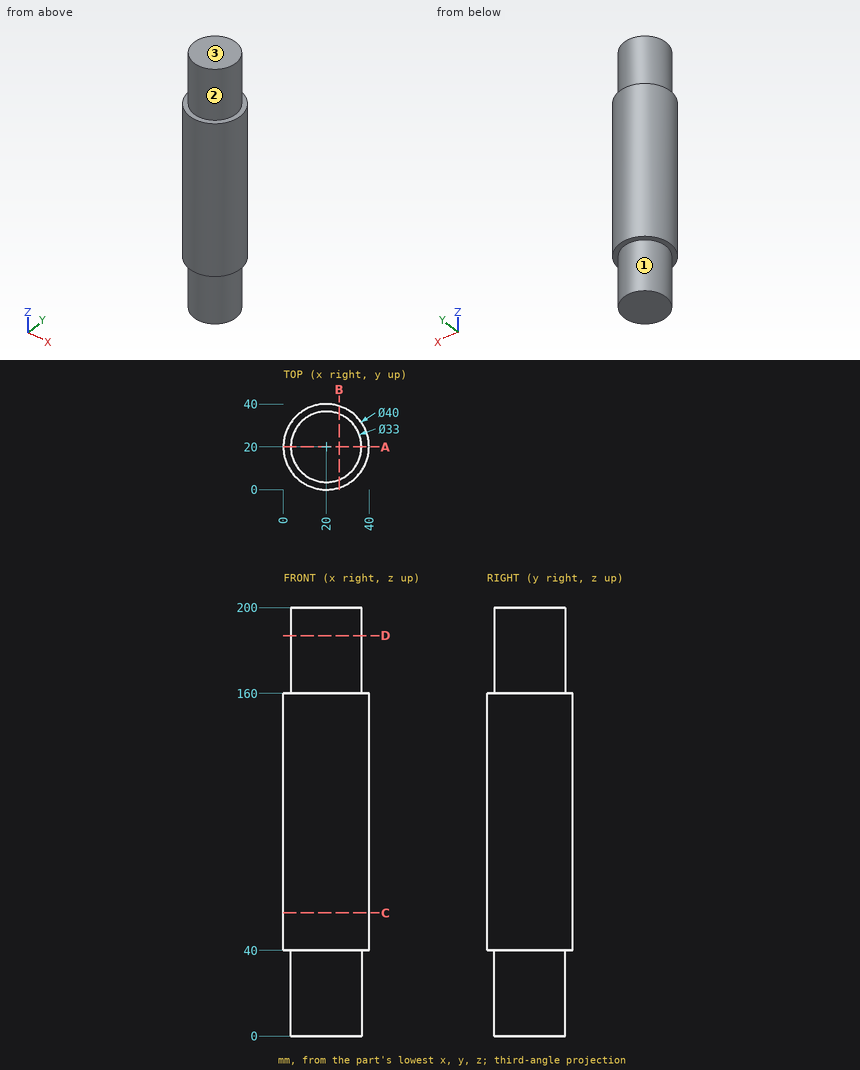
Input: dimensioned drawing with shaded views. Units: mm. Origin: part minimum x, y, z. A direction names the side the tool comes from. Round coordinates to 2 decimals unless told otherwise and drop trailing zeros. Order: outer loops, then holes, each group sorted by start corner. A loop starts at its lowest first (then second) coordinate and runs counter-clockwise, first axis right, second up. Notation, with made-up numbers: (-23, 66.5) -> (-11, 66.5) arc R28 cw to (-11, 98.5) -> close; hole circle Ø11 at (41.25, 75). An arc over 180 degrees is marked (long way). Put each result on its own line as item: value. Start each with the question number.
Q1. Reachability of the marked faces 1, 2 and 3 from +Z, -Z, +X, -X, +Y, -Y: full face, straight path, thin tool, end or side. Return the list, or none.
Q2. Section D-D on z = 187. Return the cut outline in (x, y).
Q3. Section A-A on y = 20. Return the cut outline in (x, z), and give its area (3 significant figures).
Q4. Section B-B on x = 26. Return the cut outline in (y, z), and give its area (3 significant figures).
Q5. Section C-C on z = 57.5. Return the cut outline in (x, y).
Q6. Line query: probe 1 along Y at (x, z) = (21, 118.5); probe 2 along Z at (x, y) = (20, 2.5). Output: solid intervals per line, ascending.
Q7. First-contact query: pin 1 (3 mm diameter, centred on x = 11, z = 148, fed in from -Y); pin 2 (3 mm diameter, centred on x = 36, y = 6.5, fed in from -Z); pin 3 (6 mm diameter, centred on y = 27.5, z = 43.5, fed in from +X). Flat tips, straight axial feed; report the tip coordinate or a pass-through.
Ans:
1. face 1: -Z
1. face 2: +Z
1. face 3: +Z, +X, -X, +Y, -Y
2. outline: circle Ø33 at (20, 20)
3. outline: (0, 40) -> (3.5, 40) -> (3.5, 0) -> (36.5, 0) -> (36.5, 40) -> (40, 40) -> (40, 160) -> (36.5, 160) -> (36.5, 200) -> (3.5, 200) -> (3.5, 160) -> (0, 160) -> close
3. area: 7,440 mm2
4. outline: (0.92, 40) -> (4.63, 40) -> (4.63, 0) -> (35.37, 0) -> (35.37, 40) -> (39.08, 40) -> (39.08, 160) -> (35.37, 160) -> (35.37, 200) -> (4.63, 200) -> (4.63, 160) -> (0.92, 160) -> close
4. area: 7,040 mm2
5. outline: circle Ø40 at (20, 20)
6. probe 1: y = 0.03 to 39.97
6. probe 2: z = 40 to 160
7. pin 1: stops at y = 1.46
7. pin 2: stops at z = 40
7. pin 3: stops at x = 39.49
